Input: dimensioned drawing with shaded views. Units: mm. Origin: part minimum x, y, z. A direction names the side the tool comes from. Round coordinates to 2 decimals unless told otherwise and drop trailing zeros. Loops run counter-clockwise (first coordinate to the right, second up) from the corner with the lowest first, then second, coordinate; pieces in that order, holes last.
1) Section D-D, the plane z = 7.25. Return loops of the section in (x, y).
2) Section C-C, the plane y = 3. Return loops of the section in (x, z), and give its area (3 significant figures).
3) Access query for the marked faces 1 and 2. Directions: +Z, -Z, +X, -X, +Y, -Y. A direction counts if a zero-diameter tool reaches every point of the face in a straight line with its end or side. Return the directions, or none.
4) Draft query along X for the marked faces 3, 4 and 5. Return one class per face: pulls with the +X half, pulls with the -X half, needs draft (parallel to the pull), parting line crosses it, or undercut.
5) Section B-B, the plane z = 1.75. Return loops of the section in (x, y), and give its area (3 significant figures).
6) Ray query, line 1 along Y through (x, z) = (51.5, 7.3); line 2 along X through (y, z) = (6.25, 6.75); line 3 along Z through (x, y) = (9, 2.75). Return the intervals inside material, ascending.
7) Section A-A, the plane x = 11.5. Return loops of the section in (y, z), and give its area (3 significant figures).
8) First-contact query: pin 1 (2 mm diameter, centred on x = 51.5, y = 3, fed in from +Z); pin 2 (1 mm diameter, centred on y = 5, z = 4.5, fed in from -X); pin 3 (4 mm diameter, centred on x = 38, y = 5.5, fed in from -Z). Flat tips, straight axial feed; report the tip coordinate or a pass-through.
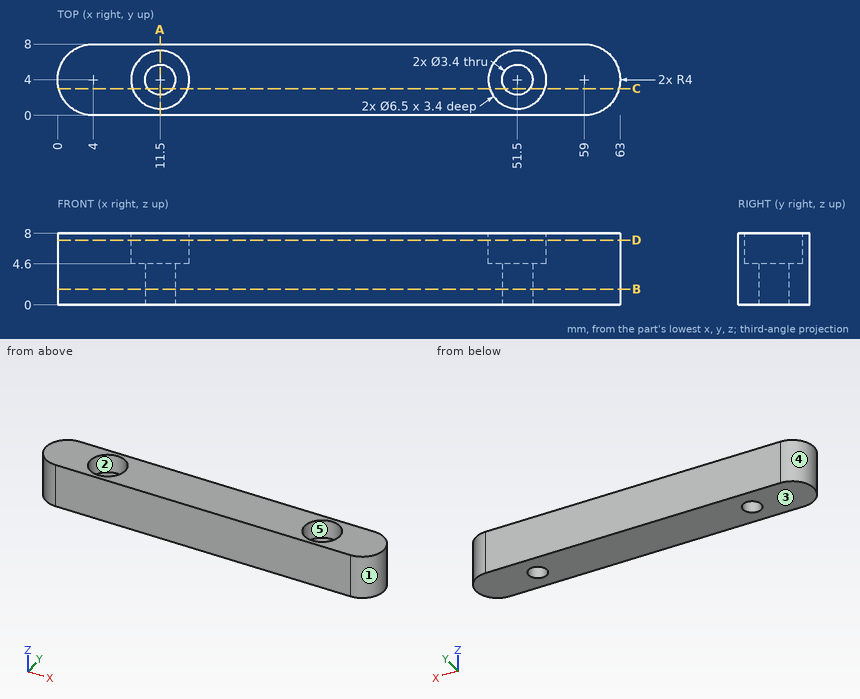
Final values:
1. outline: (4, 0) - (59, 0) arc R4 ccw to (59, 8) - (4, 8) arc R4 ccw to start; hole circle Ø6.5 at (11.5, 4); hole circle Ø6.5 at (51.5, 4)
2. outline: (0.13, 0) - (10.13, 0) - (10.13, 4.6) - (8.41, 4.6) - (8.41, 8) - (0.13, 8) - close; (12.87, 0) - (50.13, 0) - (50.13, 4.6) - (48.41, 4.6) - (48.41, 8) - (14.59, 8) - (14.59, 4.6) - (12.87, 4.6) - close; (52.87, 0) - (62.87, 0) - (62.87, 8) - (54.59, 8) - (54.59, 4.6) - (52.87, 4.6) - close
2. area: 435 mm2
3. face 1: +Z, -Z, +X
3. face 2: +Z
4. face 3: needs draft
4. face 4: pulls with the -X half
4. face 5: undercut
5. outline: (4, 0) - (59, 0) arc R4 ccw to (59, 8) - (4, 8) arc R4 ccw to start; hole circle Ø3.4 at (11.5, 4); hole circle Ø3.4 at (51.5, 4)
5. area: 472 mm2
6. line 1: y = 0 to 0.75, 7.25 to 8
6. line 2: x = 0.69 to 9.15, 13.85 to 49.15, 53.85 to 62.31
6. line 3: z = 0 to 4.6
7. outline: (0, 0) - (2.3, 0) - (2.3, 4.6) - (0.75, 4.6) - (0.75, 8) - (0, 8) - close; (5.7, 0) - (8, 0) - (8, 8) - (7.25, 8) - (7.25, 4.6) - (5.7, 4.6) - close
7. area: 26.3 mm2
8. pin 1: stops at z = 4.6
8. pin 2: stops at x = 0.03
8. pin 3: stops at z = 0
